from build123d import *

# Parameters (mm, degrees)
SKETCH1_W           = 8
SKETCH1_H           = 40
BOSS_EXTRUDE1_DEPTH = 20
CHAMFER1_SIZE       = 1
SKETCH2_R           = 3
CUT_EXTRUDE1_DEPTH  = 46.431266766


with BuildPart() as part:
    # Sketch1 → Boss-Extrude1 (new body)
    with BuildSketch(Plane(origin=(0, 0, 0), x_dir=(1, 0, 0), z_dir=(0, 1, 0))):
        with Locations((4, -20)):
            Rectangle(SKETCH1_W, SKETCH1_H)
    extrude(amount=BOSS_EXTRUDE1_DEPTH)

    # Chamfer1
    chamfer1_edges = [part.edges().sort_by_distance(p)[0] for p in [
        (0, 10, 0),
        (8, 10, 0),
        (8, 10, 40),
        (0, 10, 40),
    ]]
    chamfer(chamfer1_edges, length=CHAMFER1_SIZE)

    # Sketch2 → Cut-Extrude1 (cut, through all)
    with BuildSketch(Plane(origin=(8, 0, 0), x_dir=(0, 0, -1), z_dir=(1, 0, 0))):
        with Locations((-30, 10)):
            Circle(SKETCH2_R)
        with Locations((-10, 10)):
            Circle(SKETCH2_R)
    extrude(amount=-CUT_EXTRUDE1_DEPTH, mode=Mode.SUBTRACT)


solid = part.part
The model under review builds one solid part; all positions refer to its coordinate system, in mm. Round coordinates to 2 decimals unless told otherwise and drop trailing zeros. Loops run counter-clockwise (first coordinate to the right, second up) from the corner with the lowest first, then second, coordinate; pieces in that order, holes last. Notation, with made-up numbers: (26, 84.25) -> (62, 84.25) arc R34 cw to (62, 123.25) -> close; hole circle Ø1 at (6.25, -14). An arc over 180 degrees is marked (long way). One line per question, with ' | ' between items. Start each with the question number.
Item 1: Add section D-D, the plane z = 31. Write out the cut boundary in (x, y).
Item 2: Draft analysis for pull direction Y (two halves, no side actions). For faces 1 (the face through (4.1, 8.2, 12.4)), 2 (the face through (4, 0, 20)), 3 (the face through (0.5, 9.9, 39.5)), state which applies: +Y half, -Y half, draft (parallel to the pull), parting line (faces both ways), or undercut.
Item 3: Add section A-A, the plane z = 10. Write out the cut boundary in (x, y), then the cut area to 3 significant figures.
Item 4: Add section C-C, the plane x = 5. Write out the cut boundary in (y, z).
Item 5: Add section B-B, the plane y = 10. Write out the cut boundary in (x, z), then the cut area to 3 significant figures.
Item 6: Wall thickness on line 1 along Y through (x, z) = (4.5, 10); line 2 along Z through (x, y) = (5, 11); line 3 along Z through (x, y) = (3.5, 12.75): over which ranges is each line inside the solid? List them lowest first. Write a range as [from, to].
Return value:
1) outline: (0, 0) -> (8, 0) -> (8, 7.17) -> (0, 7.17) -> close; (0, 12.83) -> (8, 12.83) -> (8, 20) -> (0, 20) -> close
2) face 1: undercut | face 2: -Y half | face 3: draft
3) outline: (0, 0) -> (8, 0) -> (8, 7) -> (0, 7) -> close; (0, 13) -> (8, 13) -> (8, 20) -> (0, 20) -> close | area: 112 mm2
4) outline: (0, 0) -> (20, 0) -> (20, 40) -> (0, 40) -> close; hole circle Ø6 at (10, 10); hole circle Ø6 at (10, 30)
5) outline: (0, 1) -> (1, 0) -> (7, 0) -> (8, 1) -> (8, 7) -> (0, 7) -> close; (0, 13) -> (8, 13) -> (8, 27) -> (0, 27) -> close; (0, 33) -> (8, 33) -> (8, 39) -> (7, 40) -> (1, 40) -> (0, 39) -> close | area: 222 mm2
6) line 1: y = [0, 7], [13, 20] | line 2: z = [0, 7.17], [12.83, 27.17], [32.83, 40] | line 3: z = [0, 8.8], [11.2, 28.8], [31.2, 40]
